```python
from build123d import *

# Parameters (mm, degrees)
BOSS_EXTRUDE1_DEPTH = 1530
SKETCH_1_R          = 6
CUT_EXTRUDE1_DEPTH  = 1532.045394494


with BuildPart() as part:
    # Sketch1 → Boss-Extrude1 (new body)
    with BuildSketch(Plane.XY):
        with BuildLine():
            Line((0, 0), (0, 40))
            Line((0, 40), (2, 40))
            ThreePointArc((2, 40), (2.707106781, 39.707106781), (3, 39))
            Line((3, 39), (3, 8))
            ThreePointArc((3, 8), (4.464466094, 4.464466094), (8, 3))
            Line((8, 3), (39, 3))
            ThreePointArc((39, 3), (39.707106781, 2.707106781), (40, 2))
            Line((40, 2), (40, 0))
            Line((40, 0), (0, 0))
        make_face()
    extrude(amount=BOSS_EXTRUDE1_DEPTH)

    # 草图1 → Cut-Extrude1 (cut, through all)
    with BuildSketch(Plane.XZ):
        with Locations(Location((25, 1515, 0), (0, 0, 270))):
            Circle(SKETCH_1_R)
        with Locations(Location((25, 15, 0), (0, 0, 270))):
            Circle(SKETCH_1_R)
    extrude(amount=-CUT_EXTRUDE1_DEPTH, mode=Mode.SUBTRACT)


solid = part.part
```
Read the model definition and answer for the solid it produces. Units are mm, in the model's axes. A direction names the side the tool comes from. Give positions to 0.01 mm unless a question says otherwise; leave off trailing zeros. Write each loop counter-clockwise with the first axis right and the second up, starting at its lowest first coordinate (ties: lowest second). Pieces come first, ordered by that corner, then holes. Notation, with made-up numbers: (-5.75, 26) -> (24.25, 26) arc R29 cw to (24.25, 46) -> close; hole circle Ø9 at (76, 67). An arc over 180 degrees is marked (long way). Answer as a JSON object with one key per item and string values.
1) Section A-A on x = 25 is taken. Write down the section's boundary in (y, z).
Findings below:
{"outline": "(0, 0) -> (3, 0) -> (3, 9) -> (0, 9) -> close; (0, 21) -> (3, 21) -> (3, 1509) -> (0, 1509) -> close; (0, 1521) -> (3, 1521) -> (3, 1530) -> (0, 1530) -> close"}
2) Straight lines are drawn through the part: probe 1 along X at (y, z) = (1.6, 1515); probe 2 along Y at (x, z) = (17, 1350). For each, find the intervals that lie inside material, in ascending order. Write a range as from..to.
Findings below:
{"probe 1": "x = 0..19, 31..40", "probe 2": "y = 0..3"}
3) Flat-ended cylindrical pins translate along their axes: pin 1 Ø2 at (x, z) = (10.5, 1301) entering from +Y; pin 2 Ø4 at (x, z) = (4.5, 1277.5) entering from +Y; pin 3 Ø15.5 at (y, z) = (30.5, 894) entering from +X. Find the tip coordinate at first contact, or state that the pin passes through.
Findings below:
{"pin 1": "stops at y = 3", "pin 2": "stops at y = 39.87", "pin 3": "stops at x = 3"}
4) Section C-C on y = 21 is taken. Write down the section's boundary in (x, z).
Findings below:
{"outline": "(0, 0) -> (3, 0) -> (3, 1530) -> (0, 1530) -> close"}
5) Section B-B on z = 917 is taken. Write down the section's boundary in (x, y), then the cut area to 3 significant figures.
Findings below:
{"outline": "(0, 0) -> (40, 0) -> (40, 2) arc R1 ccw to (39, 3) -> (8, 3) arc R5 cw to (3, 8) -> (3, 39) arc R1 ccw to (2, 40) -> (0, 40) -> close", "area": "236 mm^2"}
6) A tool of negligible diameter and unlimited length cuts with its end or side. For faces 1 (the flat face through (0, 20, 754)), 2 (the flat face through (23, 3, 754)), from which of +Z, -Z, +X, -X, +Y, -Y can it reach the whole face along a straight path? Write none if from no direction.
Findings below:
{"face 1": "+Z, -Z, -X, +Y, -Y", "face 2": "+Z, -Z, +X, +Y"}
